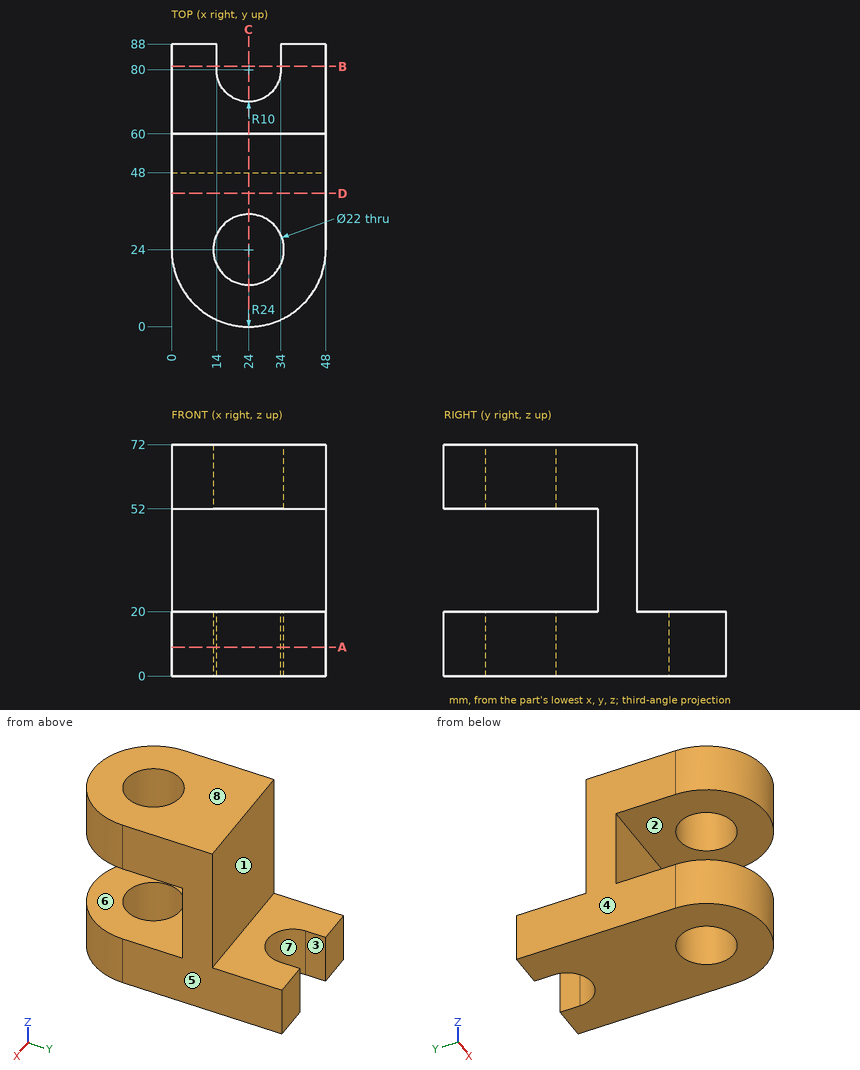
Answer from the drawing. Dimensions are ordinates in mm from the lowest x, y and z of the part. A direction names the side the tool comes from. Give positions to 0.01 mm unless a question says otherwise; leave off trailing zeros. Loops run counter-clockwise (first coordinate to the right, second up) from the corner with the lowest first, then second, coordinate; pieces in that order, holes last.
Item 1: The part is cut by section D-D (y = 41.5). Write down the section's boundary in (x, z), and give its area (3 significant figures).
Item 2: Find the intervals of material crossed by line 1 along Z through (x, y) = (45.5, 26); line 2 along X through (y, z) = (24, 60.5); line 3 along Y through (x, z) = (24, 61), in increasing order.
Item 3: The mould has two halves that part along Z. Classify the marked faces 6, 7 and 8: released by +Z, released by -Z, zero draft, split by the parting line, or undercut.
Item 4: The part is cut by section B-B (y = 81). Write down the section's boundary in (x, z), and give its area (3 significant figures).
Item 5: Each of these flat-tipped pins is pushed along its axis until it touches: pin 1 Ø20 at (x, y) = (24, 24) entering from +Z; pin 2 Ø10 at (x, z) = (31, 61.5) entering from -Y; pin 3 Ø3 at (x, z) = (15.5, 51.5) entering from -Y; pin 4 Ø5 at (x, z) = (20.5, 36.5) entering from +Y. Where does it stop, or does it pass through?
Item 6: The part is cut by section A-A (z = 9). Write down the section's boundary in (x, y), and give its area (3 significant figures).
Item 7: The part is cut by section C-C (x = 24). Write down the section's boundary in (y, z).
Item 8: For the marked faces 1, 2, 3, 4 and 5, determine the directions among +Z, -Z, +X, -X, +Y, -Y from which every point of the face is accessible in a straight line to the end or side of a thin tool.
Taken from the geometry:
1. outline: (0, 0) - (48, 0) - (48, 20) - (0, 20) - close; (0, 52) - (48, 52) - (48, 72) - (0, 72) - close
1. area: 1,920 mm2
2. line 1: z = 0 to 20, 52 to 72
2. line 2: x = 0 to 13, 35 to 48
2. line 3: y = 0 to 13, 35 to 60
3. face 6: undercut
3. face 7: zero draft
3. face 8: released by +Z
4. outline: (0, 0) - (14, 0) - (14, 20) - (0, 20) - close; (34, 0) - (48, 0) - (48, 20) - (34, 20) - close
4. area: 560 mm2
5. pin 1: passes through
5. pin 2: stops at y = 0.08
5. pin 3: stops at y = 1.07
5. pin 4: stops at y = 60
6. outline: (0, 24) arc R24 ccw to (48, 24) - (48, 88) - (34, 88) - (34, 80) arc R10 cw to (14, 80) - (14, 88) - (0, 88) - close; hole circle Ø22 at (24, 24)
6. area: 3,280 mm2
7. outline: (0, 0) - (13, 0) - (13, 20) - (0, 20) - close; (0, 52) - (13, 52) - (13, 72) - (0, 72) - close; (35, 0) - (70, 0) - (70, 20) - (60, 20) - (60, 72) - (35, 72) - (35, 52) - (48, 52) - (48, 20) - (35, 20) - close
8. face 1: +Z, +X, -X, +Y
8. face 2: +X, -X, -Y
8. face 3: +Z, -Z, +Y
8. face 4: +Z, -Z, -X, +Y, -Y
8. face 5: +Z, -Z, +X, +Y, -Y
